Drawing for the job (mm, zero at the part's lowest x, y, z). Give positions to 0.01 mm unless a question says otherwise; leave off trailing zeros. Loops run counter-clockwise (first coordinate to the right, second up) from the corner with the lowest first, then second, coordinate; pieces in that order, holes last.
1) Band-saw the part on C-C on y = 11.5. List the corners of the cut face in (x, z).
2) Two-plate mould, pull along Y, no slides. Class the marked faces 1, 2, 3 and 4: +Y half, -Y half, draft (parallel to the pull), parting line (faces both ways), or undercut.
3) Band-saw the part on A-A on x = 50. List the corners of the cut face in (y, z).
4) Band-saw the part on B-B on z = 7.5. List the corners of the cut face in (x, y).
5) Wall check: line 1 (Y direction, x = 50, z = 65); line 2 (Y direction, x = 75, z = 20); line 3 (Z direction, x = 62.5, y = 29). Give the ranges that are in metal, low to high.
6) Flat gauge pins, fed straight in: P1, Ø11, axis at y = 22.5, z = 65, coming from the -X side; P2, Ø8, axis at x = 83.5, z = 56.5, coming from the -Y side; P3, Ø3, axis at y = 29.5, z = 65, coming from the +X side; P4, Ø2, axis at x = 59.5, y = 15, coming from the -Z side. Where does each tip first touch, or does it go through?
7) Band-saw the part on D-D on x = 39. List the corners of the cut face in (y, z).
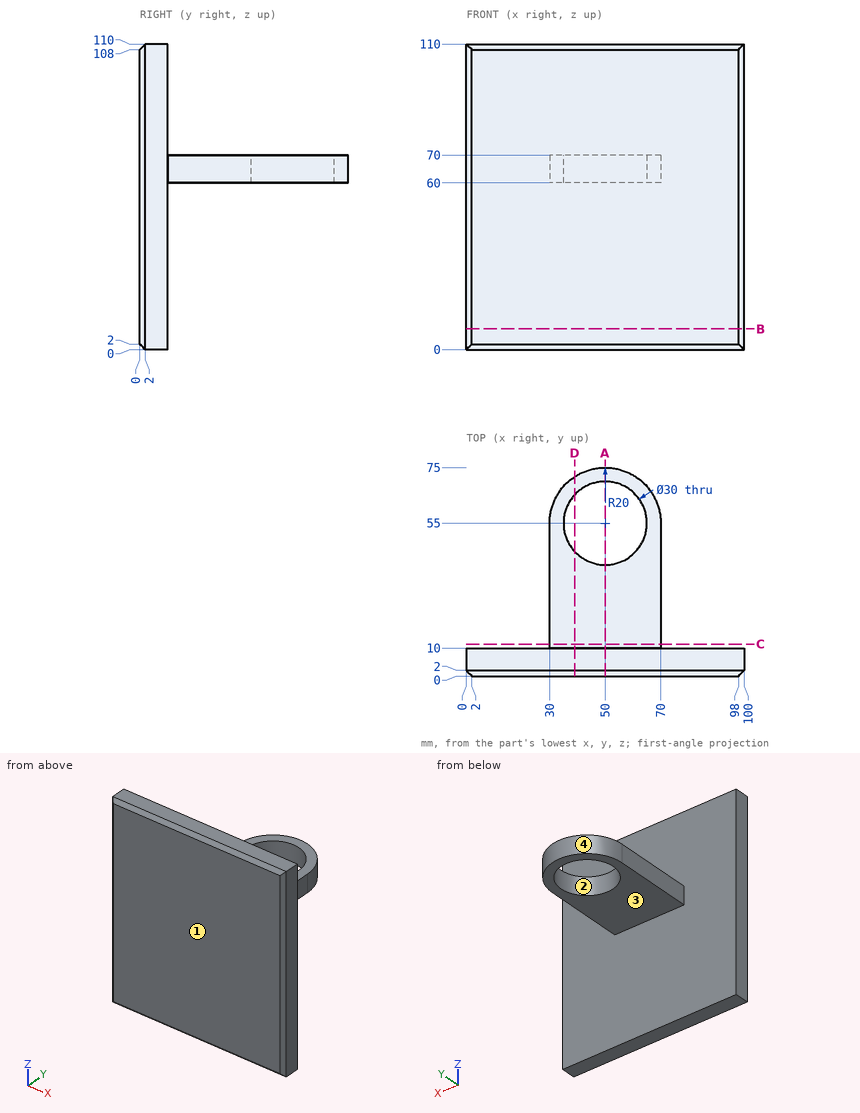
Findings below:
1. outline: (30, 60) - (70, 60) - (70, 70) - (30, 70) - close
2. face 1: -Y half
2. face 2: undercut
2. face 3: draft
2. face 4: +Y half
3. outline: (0, 2) - (2, 0) - (10, 0) - (10, 60) - (40, 60) - (40, 70) - (10, 70) - (10, 110) - (2, 110) - (0, 108) - close; (70, 60) - (75, 60) - (75, 70) - (70, 70) - close
4. outline: (0, 2) - (2, 0) - (98, 0) - (100, 2) - (100, 10) - (0, 10) - close
5. line 1: y = 0 to 40, 70 to 75
5. line 2: y = 0 to 10
5. line 3: z = 60 to 70
6. P1: stops at x = 30
6. P2: stops at y = 0
6. P3: stops at x = 70
6. P4: stops at z = 60
7. outline: (0, 2) - (2, 0) - (10, 0) - (10, 60) - (44.8, 60) - (44.8, 70) - (10, 70) - (10, 110) - (2, 110) - (0, 108) - close; (65.2, 60) - (71.7, 60) - (71.7, 70) - (65.2, 70) - close
